from build123d import *

# Parameters (mm, degrees)
HEX_BOSS_SKETCH_R                 = 32
HEX_BOSS_DEPTH                    = 24
BASE_PLATE_DEPTH                  = 24
PLATE_HOLES_SKETCH_R              = 12.5
PLATE_HOLES_2X_25_DEPTH           = 24
PLATE_HOLES_2X_25_DRAFT           = -20
PLATE_HOLES_2X_25_PROFILE_2_DEPTH = 24
PLATE_HOLES_2X_25_PROFILE_2_DRAFT = -20


with BuildPart() as part:
    # Knob Profile Sketch → Ball Knob (revolve)
    with BuildSketch(Plane.XY, mode=Mode.PRIVATE) as ball_knob_sk:
        with BuildLine():
            Line((0, 0), (0, 70))
            Line((0, 70), (23.065, 70))
            ThreePointArc((23.065, 70), (21.241041688, 59.227069146), (14.830368725, 50.37912389))
            ThreePointArc((14.830368725, 50.37912389), (10.051448448, 38.600871321), (16.770498027, 27.811075894))
            ThreePointArc((16.770498027, 27.811075894), (28.278508674, 15.969705495), (32.476230484, 0))
            Line((32.476230484, 0), (0, 0))
        make_face()
    revolve(ball_knob_sk.sketch.rotate(Axis((0, 0, 0), (0, 1, 0)), 90), axis=Axis((0, 0, 0), (0, 1, 0)))

    # Hex Boss Sketch → Hex Boss (add)
    with BuildSketch(Plane.XZ):
        Polygon((1.619817649, 49.97375502), (-38.061115187, 32.424551049), (-49.081251981, -9.541001202), (-23.142204959, -44.321984947), (20.223394412, -45.727610023), (48.360365309, -12.699412079), (40.080994757, 29.891702182), align=None)
        with Locations(Location((0, 0, 0), (0, 0, 270))):
            Circle(HEX_BOSS_SKETCH_R, mode=Mode.SUBTRACT)
    extrude(amount=HEX_BOSS_DEPTH)

    # Base Plate Sketch → Base Plate (add)
    with BuildSketch(Plane.XZ.offset(24)):
        with BuildLine():
            Line((-78, 60), (60, 60))
            Line((60, 60), (60, -60))
            Line((60, -60), (-78, -60))
            ThreePointArc((-78, -60), (-93, 0), (-78, 60))
        make_face()
    extrude(amount=BASE_PLATE_DEPTH)


with BuildPart() as plate_holes_2x_25_tool:
    # Plate Holes Sketch → Plate Holes 2xØ25 (with draft: the straight prism first)
    with BuildSketch(Plane(origin=(0, -24, 0), x_dir=(1, 0, 0), z_dir=(0, 1, 0))):
        with Locations((-67.55, 39)):
            Circle(PLATE_HOLES_SKETCH_R)
    extrude(amount=-PLATE_HOLES_2X_25_DEPTH)
    # Plate Holes 2xØ25: the draft: its side faces are tilted about the plane it starts from
    plate_holes_2x_25_sides = [plate_holes_2x_25_tool.faces().sort_by_distance(p)[0] for p in [
        (-80.05, -36, -39),
    ]]
    draft(plate_holes_2x_25_sides, Plane(origin=(0, -24, 0), x_dir=(1, 0, 0), z_dir=(0, 1, 0)), PLATE_HOLES_2X_25_DRAFT)


with BuildPart() as part_1:
    add(part.part)

    # Plate Holes 2xØ25: cut by plate_holes_2x_25_tool
    add(plate_holes_2x_25_tool.part, mode=Mode.SUBTRACT)


with BuildPart() as plate_holes_2x_25_profile_2_tool:
    # Plate Holes Sketch → Plate Holes 2xØ25 profile 2 (with draft: the straight prism first)
    with BuildSketch(Plane(origin=(0, -24, 0), x_dir=(1, 0, 0), z_dir=(0, 1, 0))):
        with Locations((-67.55, -39)):
            Circle(PLATE_HOLES_SKETCH_R)
    extrude(amount=-PLATE_HOLES_2X_25_PROFILE_2_DEPTH)
    # Plate Holes 2xØ25 profile 2: the draft: its side faces are tilted about the plane it starts from
    plate_holes_2x_25_profile_2_sides = [plate_holes_2x_25_profile_2_tool.faces().sort_by_distance(p)[0] for p in [
        (-80.05, -36, 39),
    ]]
    draft(plate_holes_2x_25_profile_2_sides, Plane(origin=(0, -24, 0), x_dir=(1, 0, 0), z_dir=(0, 1, 0)), PLATE_HOLES_2X_25_PROFILE_2_DRAFT)


with BuildPart() as part_2:
    add(part_1.part)

    # Plate Holes 2xØ25 profile 2: cut by plate_holes_2x_25_profile_2_tool
    add(plate_holes_2x_25_profile_2_tool.part, mode=Mode.SUBTRACT)


solid = part_2.part
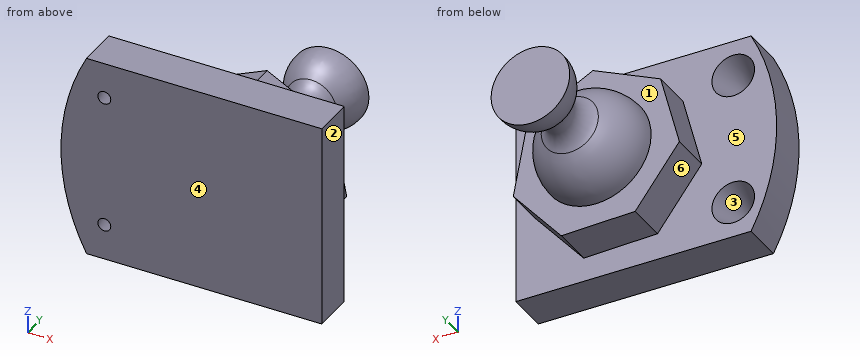
Could you check a few things on this model? Use its own coordinates, in mm. Face numbers are marked on the shaded views. A direction names the side the tool comes from. Give positions to 0.01 mm unless a question says otherwise; leave off trailing zeros. Order: outer loops, then holes, each group sorted by start corner. A loop starts at its lowest first (then second) coordinate and runs counter-clockwise, first axis right, second up.
1. Suppose I cut it at A-A (z = -39). List the corners of the cut face in (x, y) for me, plus the area to 3 significant figures.
2. I need wall thicknesses on L1, parallel to Z at x = -71.5, y = -26.5; L2, parallel to Y at x = 1.5, z = 28.5; L3, parallel to X at y = -7, z = 0. Which ranges of each line are inside material? Lowest first, please.
3. We'd pull the mould along X, two halves only. Please class the marked faces 1, 2 and 3: pulls with the +X half, pulls with the -X half, needs draft (parallel to the pull), parting line crosses it, or undercut.
4. Suppose I cut it at B-B (x = -67.55). List the corners of the cut face in (y, z) for me.
5. Suppose I cut it at C-C (x = 14). Give the number of separate pieces and of enclosed holes in the cut face, plus the area to 3 significant figures.
6. For the marked faces 4, 5 and 6, which set-ups out of +Z, -Z, +X, -X, +Y, -Y let a thin tool reach every point of the face, with its end or its side?
7. Will these pins go through, and if not, where does the flat tip stop? P1, Ø4, axis at y = -0.5, z = 10.5, coming from the -X side; P2, Ø8, axis at y = -2.5, z = 1.5, coming from the +X side; P3, Ø12, axis at x = -68, z = -47, coming from the +Y side.
Solved:
1. outline: (-86.89, -48) - (-71.31, -48) - (-80.05, -24) - (-86.89, -24) - close; (-63.79, -48) - (60, -48) - (60, -24) - (25.95, -24) - (25.95, 0) - (-27.11, 0) - (-27.11, -24) - (-55.05, -24) - close
1. area: 4,410 mm2
2. L1: z = -60 to -49.9, -28.1 to 28.1, 49.9 to 60
2. L2: y = -48 to -24, 0 to 15.5
2. L3: x = -46.58 to -32, 32 to 45.89
3. face 1: needs draft
3. face 2: pulls with the +X half
3. face 3: undercut
4. outline: (-48, -60) - (-24, -60) - (-24, -51.5) - (-48, -42.76) - close; (-48, -35.24) - (-24, -26.5) - (-24, 26.5) - (-48, 35.24) - close; (-48, 42.76) - (-24, 51.5) - (-24, 60) - (-48, 60) - close
5. separate pieces: 2
5. enclosed holes: 1
5. area: 5,590 mm2
6. face 4: +Z, -Z, +X, -X, -Y
6. face 5: +Y
6. face 6: -Z, -X, +Y
7. P1: stops at x = -44.34
7. P2: stops at x = 46.38
7. P3: stops at y = -24
